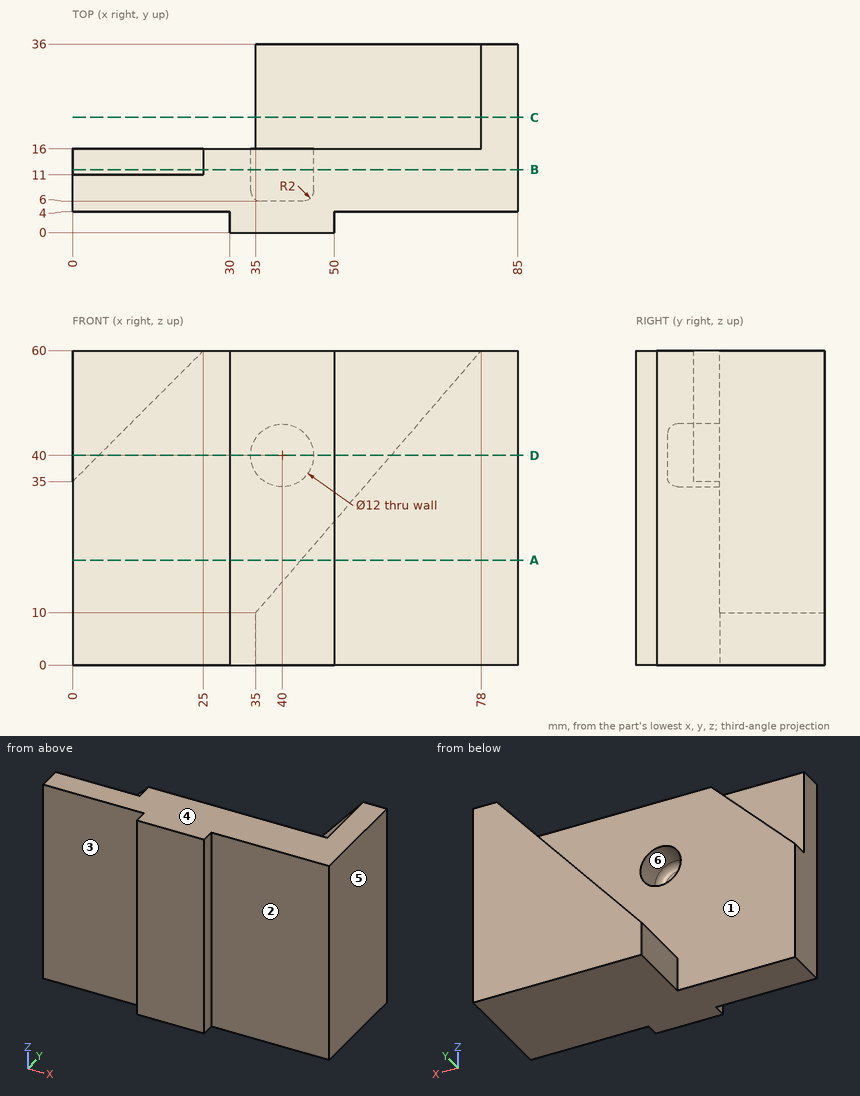
For this review, use the dimensioned drawing (mm, ordinates from the lowest corner) and the shaded views. A direction names the side the tool comes from. Coordinates: 2 decimals unless noted, no trailing zeros. Write each loop counter-clockwise with the first axis right and the second up, starting at its lowest first coordinate (ties: lowest second). Pieces come first, ordered by that corner, then holes. Notation, with made-up numbers: (59.5, 62.5) -> (106.5, 62.5) arc R36 cw to (106.5, 99.5) -> close; hole circle Ø2 at (52, 49). An arc over 180 degrees is marked (long way). Put each result on its own line as item: value.
Q1. Take a section at B-B, the plane y = 12. State the section outline as (x, z) points.
From the geometry:
outline: (0, 0) -> (85, 0) -> (85, 60) -> (25, 60) -> (0, 35) -> close; hole circle Ø12 at (40, 40)
Q2. Tool access review of the marked faces 1, 2 and 3: name each direction out of +Z, -Z, +X, -X, +Y, -Y from which nothing blocks a thin tool from reaching the whole face with its end or side.
From the geometry:
face 1: +Z, -X, +Y
face 2: +Z, -Z, +X, -Y
face 3: +Z, -Z, -X, -Y
Q3. Wall thickness on L1, parallel to Y at x = 15, z = 29; L2, parallel to Y at x = 34.5, z = 30.5; L3, parallel to X at y = 12.25, z = 40: over which ranges is each line inside the solid? List them lowest first.
From the geometry:
L1: y = 4 to 16
L2: y = 0 to 16
L3: x = 5 to 34, 46 to 85
Q4. Take a section at C-C, the plane y = 22. State the section outline as (x, z) points, then the cut area to 4 significant figures.
From the geometry:
outline: (35, 0) -> (85, 0) -> (85, 60) -> (78, 60) -> (35, 10) -> close
area: 1,925 mm2
Q5. The part is to be moulded in two halves that separate along Z. For the marked faces 4, 5 and 6, say which applies: +Z half, -Z half, draft (parallel to the pull), parting line (faces both ways), or undercut.
From the geometry:
face 4: +Z half
face 5: draft
face 6: undercut
Q6. Clearance check with flat-ended pins moving along their axes: pin 1 Ø3 at (y, z) = (29.5, 5) entering from -X; pin 2 Ø14 at (x, z) = (40, 40) entering from +Y; pin 3 Ø3 at (y, z) = (1.5, 37.5) entering from -X. State where each tip first meets the part, or that it passes through.
From the geometry:
pin 1: stops at x = 35
pin 2: stops at y = 16
pin 3: stops at x = 30
Q7. Take a section at D-D, the plane z = 40. State the section outline as (x, y) points.
From the geometry:
outline: (0, 4) -> (30, 4) -> (30, 0) -> (50, 0) -> (50, 4) -> (85, 4) -> (85, 36) -> (60.8, 36) -> (60.8, 16) -> (46, 16) -> (46, 8) arc R2 cw to (44, 6) -> (36, 6) arc R2 cw to (34, 8) -> (34, 16) -> (5, 16) -> (5, 11) -> (0, 11) -> close
Q8. Take a section at A-A, the plane z = 20. State the section outline as (x, y) points.
From the geometry:
outline: (0, 4) -> (30, 4) -> (30, 0) -> (50, 0) -> (50, 4) -> (85, 4) -> (85, 36) -> (43.6, 36) -> (43.6, 16) -> (0, 16) -> close
